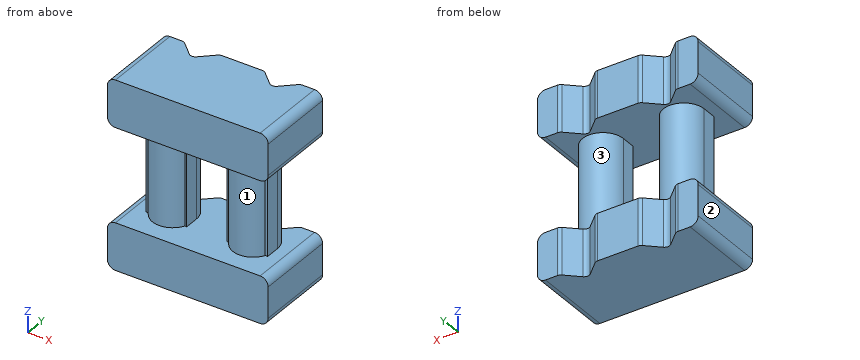
```python
from build123d import *

# Parameters (mm, degrees)
SKETCH_1_W          = 6
SKETCH_1_H          = 3
EXTRUDE_1_DEPTH     = 1.75
EXTRUDE_2_DEPTH     = 3.5
FILLET_5_R          = 0.3
FILLET_6_R          = 0.3
FILLET_7_R          = 0.3
FILLET_8_R          = 0.3
SKETCH_6_W          = 6
SKETCH_6_H          = 3
EXTRUDE_4_DEPTH     = 1.75
FILLET_9_R          = 0.3
FILLET_10_R         = 0.3
FILLET_11_R         = 0.3
FILLET_12_R         = 0.3
CUT_EXTRUDE_1_DEPTH = 10.300192295


with BuildPart() as part:
    # 草图1 → 凸台-拉伸1 (new body)
    with BuildSketch(Plane.XY):
        with Locations((-0.722891566, 3.361445783)):
            Rectangle(SKETCH_1_W, SKETCH_1_H)
    extrude(amount=EXTRUDE_1_DEPTH)

    # 草图2 → 凸台-拉伸2 (add)
    with BuildSketch(Plane(origin=(0, 0, 0), x_dir=(-1, 0, 0), z_dir=(0, 0, -1))):
        with BuildLine():
            Line((-0.097402615, 2.911445783), (-0.027108434, 2.911445783))
            Line((-0.027108434, 2.911445783), (-0.027108434, 3.451445783))
            ThreePointArc((-0.027108434, 3.451445783), (-0.787108434, 4.211445783), (-1.547108434, 3.451445783))
            Line((-1.547108434, 3.451445783), (-1.547108434, 2.911445783))
            Line((-1.547108434, 2.911445783), (-1.456814252, 2.911445783))
            ThreePointArc((-1.456814252, 2.911445783), (-0.777108434, 2.491445783), (-0.097402615, 2.911445783))
        make_face()
        with BuildLine():
            Line((1.472891566, 3.451445783), (1.472891566, 2.911445783))
            Line((1.472891566, 2.911445783), (1.543185748, 2.911445783))
            ThreePointArc((1.543185748, 2.911445783), (2.222891566, 2.491445783), (2.902597385, 2.911445783))
            Line((2.902597385, 2.911445783), (2.992891566, 2.911445783))
            Line((2.992891566, 2.911445783), (2.992891566, 3.451445783))
            ThreePointArc((2.992891566, 3.451445783), (2.232891566, 4.211445783), (1.472891566, 3.451445783))
        make_face()
    extrude(amount=EXTRUDE_2_DEPTH)

    # 圆角5
    fillet_5_edges = [part.edges().sort_by_distance(p)[0] for p in [
        (2.277108434, 3.361445783, 1.75),
    ]]
    fillet(fillet_5_edges, radius=FILLET_5_R)

    # 圆角6
    fillet_6_edges = [part.edges().sort_by_distance(p)[0] for p in [
        (2.277108434, 3.361445783, 0),
    ]]
    fillet(fillet_6_edges, radius=FILLET_6_R)

    # 圆角7
    fillet_7_edges = [part.edges().sort_by_distance(p)[0] for p in [
        (-3.722891566, 3.361445783, 1.75),
    ]]
    fillet(fillet_7_edges, radius=FILLET_7_R)

    # 圆角8
    fillet_8_edges = [part.edges().sort_by_distance(p)[0] for p in [
        (-3.722891566, 3.361445783, 0),
    ]]
    fillet(fillet_8_edges, radius=FILLET_8_R)

    # 草图6 → 凸台-拉伸4 (add)
    with BuildSketch(Plane(origin=(0, 0, -3.5), x_dir=(-1, 0, 0), z_dir=(0, 0, -1))):
        with Locations((0.722891566, 3.361445783)):
            Rectangle(SKETCH_6_W, SKETCH_6_H)
    extrude(amount=EXTRUDE_4_DEPTH)

    # 圆角9
    fillet_9_edges = [part.edges().sort_by_distance(p)[0] for p in [
        (2.277108434, 3.361445783, -5.25),
    ]]
    fillet(fillet_9_edges, radius=FILLET_9_R)

    # 圆角10
    fillet_10_edges = [part.edges().sort_by_distance(p)[0] for p in [
        (2.277108434, 3.361445783, -3.5),
    ]]
    fillet(fillet_10_edges, radius=FILLET_10_R)

    # 圆角11
    fillet_11_edges = [part.edges().sort_by_distance(p)[0] for p in [
        (-3.722891566, 3.361445783, -5.25),
    ]]
    fillet(fillet_11_edges, radius=FILLET_11_R)

    # 圆角12
    fillet_12_edges = [part.edges().sort_by_distance(p)[0] for p in [
        (-3.722891566, 3.361445783, -3.5),
    ]]
    fillet(fillet_12_edges, radius=FILLET_12_R)

    # 草图7 → 切除-拉伸1 (cut, through all)
    with BuildSketch(Plane.XY.offset(1.75)):
        with BuildLine():
            Line((-2.972891566, 4.861445783), (-1.472891566, 4.861445783))
            ThreePointArc((-1.472891566, 4.861445783), (-1.545812961, 4.847678085), (-1.608694758, 4.808270485))
            Line((-1.608694758, 4.808270485), (-2.088349842, 4.364621081))
            ThreePointArc((-2.088349842, 4.364621081), (-2.224416187, 4.311445956), (-2.360342129, 4.36497896))
            Line((-2.360342129, 4.36497896), (-2.836702471, 4.807912606))
            ThreePointArc((-2.836702471, 4.807912606), (-2.899725196, 4.847581976), (-2.972891566, 4.861445783))
        make_face()
        with BuildLine():
            Line((0.162911626, 4.808270485), (0.642566709, 4.364621081))
            ThreePointArc((0.642566709, 4.364621081), (0.778633055, 4.311445956), (0.914558997, 4.36497896))
            Line((0.914558997, 4.36497896), (1.390919338, 4.807912606))
            ThreePointArc((1.390919338, 4.807912606), (1.453942064, 4.847581976), (1.527108434, 4.861445783))
            Line((1.527108434, 4.861445783), (0.027108434, 4.861445783))
            ThreePointArc((0.027108434, 4.861445783), (0.100029829, 4.847678085), (0.162911626, 4.808270485))
        make_face()
    extrude(amount=-CUT_EXTRUDE_1_DEPTH, mode=Mode.SUBTRACT)


solid = part.part
```
Verification items for the finished model (mm, model axes). Face numbers are marked on the shaded views. A direction names the side the tool comes from. Give positions to 0.01 mm unless a question says otherwise; leave off trailing zeros. Order: outer loops, then holes, each group sorted by start corner. A loop starts at its lowest first (then second) coordinate and runs counter-clockwise, first axis right, second up. Notation, with made-up numbers: (29, 70) -> (78, 70) arc R20 cw to (78, 83) -> close; hole circle Ø3 at (-36, 40.25). An arc over 180 degrees is marked (long way). One line per item, written item: value.
(1) Sectioned sample at A-A on y = 2.25. Record the cut outline in (x, z).
Final values:
outline: (-3.72, -4.95) arc R0.3 ccw to (-3.42, -5.25) -> (1.98, -5.25) arc R0.3 ccw to (2.28, -4.95) -> (2.28, -3.8) arc R0.3 ccw to (1.98, -3.5) -> (-3.42, -3.5) arc R0.3 ccw to (-3.72, -3.8) -> close; (-3.72, 0.3) arc R0.3 ccw to (-3.42, 0) -> (1.98, 0) arc R0.3 ccw to (2.28, 0.3) -> (2.28, 1.45) arc R0.3 ccw to (1.98, 1.75) -> (-3.42, 1.75) arc R0.3 ccw to (-3.72, 1.45) -> close
(2) Scan lines: line 1 along Z through (x, y) = (-3, 4.05); line 2 along X through (y, z) = (3.45, -2.25); line 3 along Y through (x, z) = (0.8, 0.25). Record each from-to range of solid material in increasing order. Write a range as [from, to].
Final values:
line 1: [-5.25, -3.5], [0, 1.75]
line 2: [-2.99, -1.47], [0.03, 1.55]
line 3: [1.86, 4.31]
(3) Sectioned sample at B-B on z = -1.25. Record the cut outline in (x, y).
Final values:
outline: (-2.99, 2.91) -> (-2.9, 2.91) arc R0.76 ccw to (-1.54, 2.91) -> (-1.47, 2.91) -> (-1.47, 3.45) arc R0.76 ccw to (-2.99, 3.45) -> close; (0.03, 2.91) -> (0.1, 2.91) arc R0.76 ccw to (1.46, 2.91) -> (1.55, 2.91) -> (1.55, 3.45) arc R0.76 ccw to (0.03, 3.45) -> close
(4) Sectioned sample at C-C on x = 1.65. Record the cut outline in (y, z).
Final values:
outline: (1.86, -5.25) -> (4.86, -5.25) -> (4.86, -3.5) -> (1.86, -3.5) -> close; (1.86, 0) -> (4.86, 0) -> (4.86, 1.75) -> (1.86, 1.75) -> close
(5) Tool access check on the marked faces 1, 2 and 3. Record the directions out of +Z, -Z, +X, -X, +Y, -Y that give a thin tool (end or side, any length) a straight path to the whole face; none if there is none.
Final values:
face 1: -Y
face 2: +Z, -Z, -X, +Y, -Y
face 3: +Y
(6) Sectioned sample at D-D on z = -4.5. Record the cut outline in (x, y), then the cut area to 3 significant figures.
Final values:
outline: (-3.72, 1.86) -> (2.28, 1.86) -> (2.28, 4.86) -> (1.53, 4.86) arc R0.2 ccw to (1.39, 4.81) -> (0.91, 4.36) arc R0.2 cw to (0.64, 4.36) -> (0.16, 4.81) arc R0.2 ccw to (0.03, 4.86) -> (-1.47, 4.86) arc R0.2 ccw to (-1.61, 4.81) -> (-2.09, 4.36) arc R0.2 cw to (-2.36, 4.36) -> (-2.84, 4.81) arc R0.2 ccw to (-2.97, 4.86) -> (-3.72, 4.86) -> close
area: 17.2 mm^2
